Input: part model. Units: mm. Frame: model coordinates. A direction names the side the tool comes from. Give positions to 0.01 mm unless a question says otherwise; leave off trailing zeros. Write each loop counter-clockwise with the first axis right and the second up, starting at its lowest first coordinate (ties: lowest second). Pieces come first, ordered by that corner, then holes. Notation, with made-up numbers: (-2, 49.5) -> (38, 49.5) arc R19 cw to (38, 86.5) -> close; hole circle Ø6 at (85.25, 30.25). An arc over 180 degrees is marked (long way). Return JSON: item names as keys, results as strings. Group by question number.
Item 1: Pin query (flat end, axial travel): P1, Ø3, axis at x = 15, y = -4, coming from the -Z side; P2, Ø4, axis at x = 14, z = -5, coming from the -Y side; P3, Ø1, axis at x = -20.5, z = -2, coming from the +Y side. Return the tip coordinate at first contact, or that it passes through.
Item 2: Set-up query: faces 4 (the face through (19.05, 5, 2)), 5 (the face through (-26.81, 3.86, 5.04)). Return all of +Z, -Z, +X, -X, +Y, -Y with unobstructed straight access to the full face (end or side cutting, diameter ignored); none if empty.
Item 3: Line query: line 1 (X direction, y = -0.5, z = -5) (3 decimals); line 2 (Y direction, x = 14, z = -0.25); line 3 (Y direction, x = -30, z = 3). Output: solid intervals per line, ascending. Write a range as [from, to].
Item 4: Section A-A, the plane x = -18. Return loops of the section in (y, z).
Item 5: Mould query, pull axis X, two halves, no side actions, for faces 1 (the face through (14.29, 3.86, 5.04)), 2 (the face through (44.45, 0, 0)), 3 (the face through (6.985, 5, 2)). Classes: released by +X, released by -X, zero draft, split by the parting line, or undercut.
from build123d import *


with BuildPart() as part:
    # Rod Half-Profile Sketch → Grooved Rod Revolve (revolve)
    with BuildSketch(Plane.XY, mode=Mode.PRIVATE) as grooved_rod_revolve_sk:
        Polygon((-44.45, 0), (-44.45, 6.35), (-9.652, 6.35), (-9.652, 4.953), (-7.239, 4.953), (-7.239, 6.35), (-2.413, 6.35), (-2.413, 4.953), (0, 4.953), (0, 6.35), (6.985, 6.35), (6.985, 4.953), (9.398, 4.953), (9.398, 6.35), (19.05, 6.35), (19.05, 4.953), (21.463, 4.953), (21.463, 6.35), (44.45, 6.35), (44.45, 0), align=None)
    revolve(grooved_rod_revolve_sk.sketch.rotate(Axis((49.991353887, 0, 0), (-1, 0, 0)), 90), axis=Axis((49.991353887, 0, 0), (-1, 0, 0)))


solid = part.part
Answer below:
{
 "1": {"P1": "stops at z = -5.84", "P2": "stops at y = -5.6", "P3": "stops at y = 6.17"},
 "2": {"face 4": "none", "face 5": "+X, -X"},
 "3": {"line 1": "x = [-44.45, -9.652], [-7.239, -2.413], [0, 6.985], [9.398, 19.05], [21.463, 44.45]", "line 2": "y = [-6.35, 6.35]", "line 3": "y = [-5.6, 5.6]"},
 "4": {"outline": "circle Ø12.7 at (0, 0)"},
 "5": {"face 1": "zero draft", "face 2": "released by +X", "face 3": "undercut"}
}
